The model under review builds one solid part; all positions refer to its coordinate system, in mm. Face numbers are marked on the shaded views. Give positions to 0.01 mm unless a question says otherwise; leave off trailing zeros. Order: outer loops, then holes, each group sorted by start corner. A loop starts at its lowest first (then second) coordinate and runs counter-clockwise, first axis right, second up. Notation, with made-up numbers: (-39, -16) - (-33, -16) arc R22 ccw to (-33, 16) - close; hole circle Ø11 at (89.25, 77). An arc over 180 degrees is marked (long way). Use a Markdown table: item, result. Add a question column.
```python
from build123d import *

# Parameters (mm, degrees)
SKETCH_1_W              = 36
SKETCH_1_H              = 36
EXTRUDE_1_DEPTH         = 4
CHAMFER_1_SIZE          = 10
HOLE_WIZARD_10_0_10_1_D = 10


with BuildPart() as part:
    # 草图1 → 凸台-拉伸1 (new body)
    with BuildSketch(Plane.XY):
        with Locations((18, 18)):
            Rectangle(SKETCH_1_W, SKETCH_1_H)
    extrude(amount=EXTRUDE_1_DEPTH)

    # 倒角1
    chamfer_1_edges = [part.edges().sort_by_distance(p)[0] for p in [
        (0, 36, 2),
    ]]
    chamfer(chamfer_1_edges, length=CHAMFER_1_SIZE)

    # Ø10.0 (10) 直径孔1 (through all)
    with Locations(Plane.XY.offset(4)):
        with Locations((21, 15)):
            Hole(HOLE_WIZARD_10_0_10_1_D / 2)


solid = part.part
```
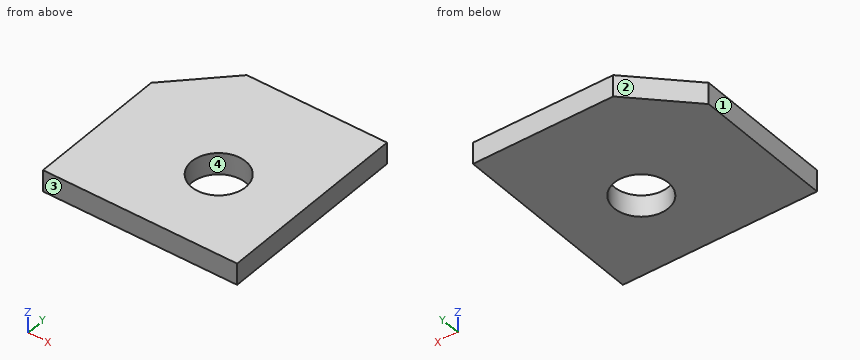
Q1. Clearance check with a flat-ended pin moving along its axis: P1, Ø1, axis at y = 28.5, z = 2, coming from the -X side. State where the tip first meets the part, or that it passes through.
Q2. Wall thickness on probe 1 along Y at (x, z) = (21, 1.55); probe 2 along X at (y, z) = (11, 2.35); probe 3 along Y at (x, z) = (23, 2.75): over which ranges is each line inside the solid? List them lowest first.
Q3. We need section A-A (x = 17). Write out the cut boundary in (y, z).
Q4. We need section B-B (y = 12). Write out the cut boundary in (x, z).
Q5. We need section C-C (z = 2.35). Write out the cut boundary in (x, y), plus the area to 3 significant figures.
Q6. We need section D-D (y = 31). Write out the cut boundary in (x, z), plus the area to 3 significant figures.
Q7. Draft analysis for pull direction Y (two halves, no side actions). For the marked faces 1, 2, 3 and 4, state which applies: pulls with the +Y half, pulls with the -Y half, needs draft (parallel to the pull), parting line crosses it, or undercut.
Here are the results:
| question | item | result |
|---|---|---|
| 1 | P1 | x = 2 |
| 2 | probe 1 | 0 to 10, 20 to 36 |
| 2 | probe 2 | 0 to 18, 24 to 36 |
| 2 | probe 3 | 0 to 10.42, 19.58 to 36 |
| 3 | outline | (0, 0) - (12, 0) - (12, 4) - (0, 4) - close; (18, 0) - (36, 0) - (36, 4) - (18, 4) - close |
| 4 | outline | (0, 0) - (17, 0) - (17, 4) - (0, 4) - close; (25, 0) - (36, 0) - (36, 4) - (25, 4) - close |
| 5 | outline | (0, 0) - (36, 0) - (36, 36) - (10, 36) - (0, 26) - close; hole circle Ø10 at (21, 15) |
| 5 | area | 1,170 mm2 |
| 6 | outline | (5, 0) - (36, 0) - (36, 4) - (5, 4) - close |
| 6 | area | 124 mm2 |
| 7 | face 1 | needs draft |
| 7 | face 2 | pulls with the +Y half |
| 7 | face 3 | pulls with the -Y half |
| 7 | face 4 | undercut |
